For this review, take the finished solid that the model builds, in its own axes (mm). Face numbers are marked on the shaded views. A direction names the side the tool comes from. Coordinates: 2 decimals unless noted, no trailing zeros. Loops run counter-clockwise (first coordinate to the right, second up) from the corner with the lowest first, then second, coordinate; pieces in that order, holes last. Notation, with made-up numbers: M 48,68.25 L 95,68.25 A20 ccw 95,96.25 Z; hole C 68,59 d8. An arc over 180 degrees is marked long. Write each question's results on one line, items separated by ' | '. Start each with the question number.
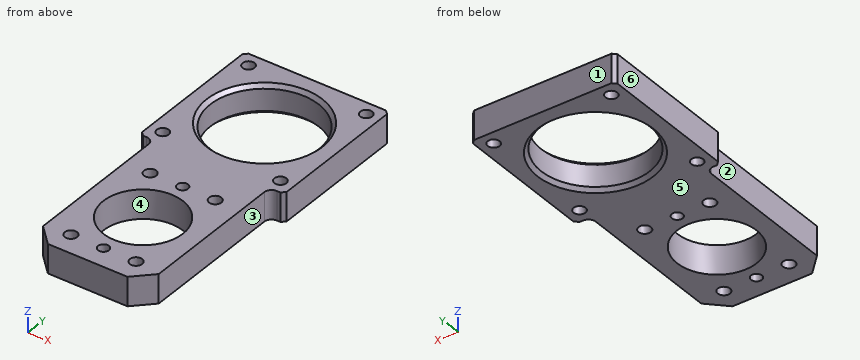
```python
from build123d import *

# Parameters (mm, degrees)
BOSS_EXTRUDE1_DEPTH  = 4
M4_TAPPED_HOLE1_D    = 3.3
M3_CLEARANCE_HOLE1_D = 3.4
SKETCH6_R            = 15
SKETCH6_R_2          = 1.5
SKETCH6_R_3          = 11
CUT_EXTRUDE1_DEPTH   = 49.541219597
CHAMFER1_SIZE        = 5
CHAMFER2_SIZE        = 1
FILLET1_R            = 2


with BuildPart() as part:
    # Sketch1 → Boss-Extrude1 (new, symmetric)
    with BuildSketch(Plane.XY):
        Polygon((-16, 3.5), (-16, -43.5), (16, -43.5), (16, 3.5), (20, 3.5), (20, 43.5), (-20, 43.5), (-20, 3.5), align=None)
    extrude(amount=BOSS_EXTRUDE1_DEPTH, both=True)

    # M4 Tapped Hole1 (through all)
    with Locations(Plane.XY.offset(4)):
        with Locations((-16.263455967, 39.763455967), (16.263455967, 39.763455967), (16.263455967, 7.236544033), (-16.263455967, 7.236544033)):
            Hole(M4_TAPPED_HOLE1_D / 2)

    # M3 Clearance Hole1 (through all)
    with Locations(Plane.XY.offset(4)):
        with Locations((-9, -7.5), (9, -7.5), (9, -37.5), (-9, -37.5)):
            Hole(M3_CLEARANCE_HOLE1_D / 2)

    # Sketch6 → Cut-Extrude1 (cut, through all)
    with BuildSketch(Plane.XY.offset(4)):
        with Locations((0, 23.5)):
            Circle(SKETCH6_R)
        with Locations((0, -7.5)):
            Circle(SKETCH6_R_2)
        with Locations((0, -37.5)):
            Circle(SKETCH6_R_2)
        with Locations((0, -22.5)):
            Circle(SKETCH6_R_3)
    extrude(amount=-CUT_EXTRUDE1_DEPTH, mode=Mode.SUBTRACT)

    # Chamfer1
    chamfer1_edges = [part.edges().sort_by_distance(p)[0] for p in [
        (16, -43.5, 0),
        (-16, -43.5, 0),
    ]]
    chamfer(chamfer1_edges, length=CHAMFER1_SIZE)

    # Chamfer2
    chamfer2_edges = [part.edges().sort_by_distance(p)[0] for p in [
        (-20, 3.5, 0),
        (-20, 43.5, 0),
        (20, 43.5, 0),
        (20, 3.5, 0),
        (-15, 23.5, -4),
        (-15, 23.5, 4),
    ]]
    chamfer(chamfer2_edges, length=CHAMFER2_SIZE)

    # Fillet1
    fillet1_edges = [part.edges().sort_by_distance(p)[0] for p in [
        (-16, 3.5, 0),
        (16, 3.5, 0),
    ]]
    fillet(fillet1_edges, radius=FILLET1_R)


solid = part.part
```
Q1. Take a section at C-C, the plane y = -22.5. Give the boundary of the cut face in (x, z), then the cut area to 3 significant figures.
Q2. Take a section at A-A, the plane x = 0. Give the boundary of the cut face in (y, z), then the cut area to 3 significant figures.
Q3. For the marked faces 1, 2 and 3, list the 3-axis set-ups (+Z, -Z, +X, -X, +Y, -Y) from which the entire face can be reached by the end or side of a thin tool; tool diameter is ignored.
Q4. The part is to be moulded in two halves that separate along X. For the marked faces 4, 5 and 6, say which applies: pulls with the +X half, pulls with the -X half, needs draft (parallel to the pull), parting line crosses it, or undercut.
Q5. Insertion check: P1, Ø0.5, axis at x = 18.5, z = 0, coming from the -Y side; P2, Ø4, axis at y = -11, z = 1.5, coming from the -X side; P3, Ø4, axis at y = -3.5, z = -1.5, coming from the +X side. Each pin has a flat end and moves straight along its axis. Give the tip position at first contact, or say it passes through.
Q6. Take a section at D-D, the plane z = 2. Give the number of separate pieces and of enclosed holes in the cut face, then the cut area to 3 significant figures.
Q7. Take a section at B-B, the plane y = -7.5. Give the boundary of the cut face in (x, z), then the cut area to 3 significant figures.
Q8. To check wall thickness, follow line 1 along Y through (x, z) = (0, 0.85); line 2 along Y through (x, z) = (8, -3.25); line 3 along X through (y, z) = (6, -1.25). State the ranges of each line that lie inside material, in increasing order.
Results:
1) outline: M -16,-4 L -11,-4 L -11,4 L -16,4 Z; M 11,-4 L 16,-4 L 16,4 L 11,4 Z | area: 80.0 mm^2
2) outline: M -43.5,-4 L -39,-4 L -39,4 L -43.5,4 Z; M -36,-4 L -33.5,-4 L -33.5,4 L -36,4 Z; M -11.5,-4 L -9,-4 L -9,4 L -11.5,4 Z; M -6,-4 L 7.5,-4 L 8.5,-3 L 8.5,3 L 7.5,4 L -6,4 Z; M 38.5,-3 L 39.5,-4 L 43.5,-4 L 43.5,4 L 39.5,4 L 38.5,3 Z | area: 230 mm^2
3) face 1: +Z, -Z, +X, -X, +Y | face 2: +Z, -Z, -X, -Y | face 3: +Z, -Z, +X, -Y
4) face 4: undercut | face 5: needs draft | face 6: pulls with the -X half
5) P1: y = 3.5 | P2: x = -16 | P3: x = 16
6) separate pieces: 1 | enclosed holes: 12 | area: 1,910 mm^2
7) outline: M -16,-4 L -10.7,-4 L -10.7,4 L -16,4 Z; M -7.3,-4 L -1.5,-4 L -1.5,4 L -7.3,4 Z; M 1.5,-4 L 7.3,-4 L 7.3,4 L 1.5,4 Z; M 10.7,-4 L 16,-4 L 16,4 L 10.7,4 Z | area: 178 mm^2
8) line 1: -43.5 to -39, -36 to -33.5, -11.5 to -9, -6 to 8.5, 38.5 to 43.5 | line 2: -43.5 to -38.87, -36.13 to -30.05, -14.95 to -8.87, -6.13 to 10.52, 36.48 to 43.5 | line 3: -20 to -17.36, -15.17 to 15.17, 17.36 to 20
